Verification items for the finished model (mm, model axes). A direction names the side the tool comes from. Round coordinates to 2 decimals unless told otherwise and drop trailing zeros. Loops run counter-clockwise (first coordinate to the right, second up) from the corner with the lowest first, then second, coordinate; pieces in that order, holes last. Notation, with made-up numbers: (19.5, 54) -> (37.5, 54) arc R27 cw to (37.5, 88) -> close; hole circle Ø10 at (-33.75, 9). An arc over 180 degrees is marked (long way). Write item = value, one per line.
```python
from build123d import *

# Parameters (mm, degrees)
SKETCH1_R           = 3
BOSS_EXTRUDE1_DEPTH = 12
SKETCH2_R           = 7.5
BOSS_EXTRUDE2_DEPTH = 10
SKETCH3_R           = 12.5
BOSS_EXTRUDE3_DEPTH = 15
CUT_EXTRUDE1_DEPTH  = 8


with BuildPart() as part:
    # Sketch1 → Boss-Extrude1 (new body)
    with BuildSketch(Plane(origin=(0, 0, 0), x_dir=(1, 0, 0), z_dir=(0, 1, 0))):
        with Locations(Location((0, 0, 0), (0, 0, 270))):
            Circle(SKETCH1_R)
    extrude(amount=BOSS_EXTRUDE1_DEPTH)

    # Sketch2 → Boss-Extrude2 (add)
    with BuildSketch(Plane(origin=(0, 12, 0), x_dir=(1, 0, 0), z_dir=(0, 1, 0))):
        with Locations(Location((0, 0, 0), (0, 0, 270))):
            Circle(SKETCH2_R)
    extrude(amount=BOSS_EXTRUDE2_DEPTH)

    # Sketch3 → Boss-Extrude3 (add)
    with BuildSketch(Plane(origin=(0, 22, 0), x_dir=(1, 0, 0), z_dir=(0, 1, 0))):
        with Locations(Location((0, 0, 0), (0, 0, 270))):
            Circle(SKETCH3_R)
    extrude(amount=BOSS_EXTRUDE3_DEPTH)

    # Sketch4 → Cut-Extrude1 (cut)
    with BuildSketch(Plane(origin=(0, 37, 0), x_dir=(1, 0, 0), z_dir=(0, 1, 0))):
        Polygon((0, 8.660254038), (-7.5, 4.330127019), (-7.5, -4.330127019), (0, -8.660254038), (7.5, -4.330127019), (7.5, 4.330127019), align=None)
    extrude(amount=-CUT_EXTRUDE1_DEPTH, mode=Mode.SUBTRACT)


solid = part.part
```
(1) Set-up check for faces 1 (the face through (-7.5, 33, 0)), 2 (the face through (0.1, 12, 3.2)), 3 (the face through (3.755, 29.395, 11.923)): record each of +Z, -Z, +X, -X, +Y, -Y from which the full face is reachable in a straight line by a thin tool's end or side.
Filled sheet:
face_1 = +Y
face_2 = -Y
face_3 = +Y, -Y
(2) Sectioned sample at A-A, the plane y = 34. Record the cut outline in (x, z), and give its area (3 significant figures).
Filled sheet:
outline = circle Ø25 at (0, 0); hole (-7.5, -4.33) -> (0, -8.66) -> (7.5, -4.33) -> (7.5, 4.33) -> (0, 8.66) -> (-7.5, 4.33) -> close
area = 296 mm2
(3) Go/stop test with flat-tipped pins: pin 1 Ø4 at (x, z) = (-4.5, 9) entering from -Y; pin 2 Ø10 at (y, z) = (28.5, 4) entering from -X; pin 3 Ø10 at (y, z) = (19.5, 7.5) entering from +X; pin 4 Ø8 at (x, y) = (-5, 10.5) entering from +Z. Record where each tip stops, or that it passes through.
Filled sheet:
pin_1 = 22
pin_2 = -12.5
pin_3 = 12.09
pin_4 = 7.39
(4) Sectioned sample at D-D, the plane y = 9.5. Record the cut outline in (x, z), and give its area (3 significant figures).
Filled sheet:
outline = circle Ø6 at (0, 0)
area = 28.3 mm2
(5) Sectioned sample at B-B, the plane z = 0. Record the cut outline in (x, y).
Filled sheet:
outline = (-12.5, 22) -> (-7.5, 22) -> (-7.5, 12) -> (-3, 12) -> (-3, 0) -> (3, 0) -> (3, 12) -> (7.5, 12) -> (7.5, 22) -> (12.5, 22) -> (12.5, 37) -> (7.5, 37) -> (7.5, 29) -> (-7.5, 29) -> (-7.5, 37) -> (-12.5, 37) -> close
(6) Sectioned sample at C-C, the plane x = 7. Record the cut outline in (y, z), and give its area (3 significant figures).
Filled sheet:
outline = (12, -2.69) -> (22, -2.69) -> (22, -10.36) -> (37, -10.36) -> (37, -4.62) -> (29, -4.62) -> (29, 4.62) -> (37, 4.62) -> (37, 10.36) -> (22, 10.36) -> (22, 2.69) -> (12, 2.69) -> close
area = 291 mm2
(7) Material ranges on probe 1 along Y at (x, z) = (-4.75, 7); probe 2 along X at (y, z) = (34.5, 6.5); probe 3 along Y at (x, z) = (-4.75, 2.5), recorded low to high. Write a range as from..to.
Filled sheet:
probe_1 = 22..37
probe_2 = -10.68..-3.74, 3.74..10.68
probe_3 = 12..29
(8) Draft check along Z on faces 4 (the face through (0.33, 16.93, -7.493)), 5 (the face through (0, 0, 0)), 6 (the face through (-3.698, 33.056, -6.526)). Enter one of: released by +Z, released by -Z, zero draft, split by the parting line, or undercut.
Filled sheet:
face_4 = split by the parting line
face_5 = zero draft
face_6 = undercut
